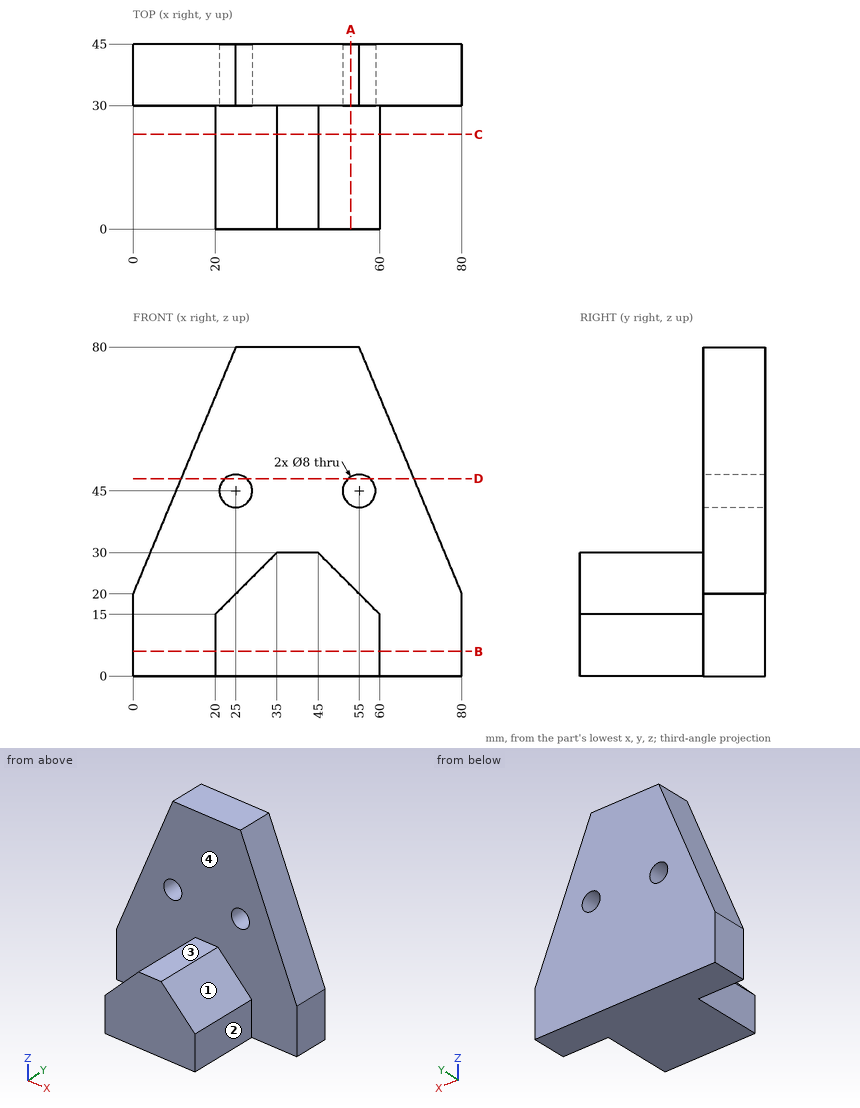
Study the drawing (mm; zero at the part's minimum x, y, z) and answer. A direction names the side the tool comes from. Round coordinates to 2 decimals unless told otherwise and drop trailing zeros. Order: outer loops, then holes, each group sorted by start corner. A loop starts at its lowest first (then second) coordinate and runs counter-clockwise, first axis right, second up. Notation, with made-up numbers: M 14.5,-39.5 L 47.5,-39.5 A24 cw 47.5,-11.5 Z; hole C 79.5,78.5 d9. An arc over 180 degrees is marked long. One line per item, written item: value.
Q1. For the marked faces 1, 2, 3 and 4, determine the directions among +Z, -Z, +X, -X, +Y, -Y from which every point of the face is accessible in a straight line to the end or side of a thin tool.
Derived:
face 1: +Z, +X, -Y
face 2: +Z, -Z, +X, -Y
face 3: +Z, +X, -X, -Y
face 4: +Z, -Y
Q2. Find section C-C on y = 23. Write down the section's boundary in (x, z).
Derived:
outline: M 20,0 L 60,0 L 60,15 L 45,30 L 35,30 L 20,15 Z
Q3. Find section D-D on z = 48. Write down the section's boundary in (x, y), then the cut area to 3 significant figures.
Derived:
outline: M 11.67,30 L 22.35,30 L 22.35,45 L 11.67,45 Z; M 27.65,30 L 52.35,30 L 52.35,45 L 27.65,45 Z; M 57.65,30 L 68.33,30 L 68.33,45 L 57.65,45 Z
area: 691 mm²
Q4. Flat-ended cylindrical pins translate along their axes: pin 1 (24 mm diameter, centred on x = 26, z = 57, fed in from -Y); pin 2 (4.5 mm diameter, centred on y = 8, z = 9.5, fed in from +X); pin 3 (4.5 mm diameter, centred on y = 8.5, z = 5.5, fed in from -X). Find the tip coordinate at first contact, or state that the pin passes through.
Derived:
pin 1: y = 30
pin 2: x = 60
pin 3: x = 20
Q5. Find section A-A on x = 53. Write down the section's boundary in (y, z).
Derived:
outline: M 0,0 L 45,0 L 45,41.54 L 30,41.54 L 30,22 L 0,22 Z; M 30,48.46 L 45,48.46 L 45,80 L 30,80 Z
Q6. Straight lines are drawn through the part: line 1 (X direction, y = 35, z = 45); line 2 (Y direction, x = 76, z = 5.5); line 3 (X direction, y = 9, z = 9). For each, find the intervals that lie inside material, in ascending order.
Derived:
line 1: 10.42 to 21, 29 to 51, 59 to 69.58
line 2: 30 to 45
line 3: 20 to 60
Q7. Find section B-B on z = 6. Write down the section's boundary in (x, y), then the cut area to 3 significant figures.
Derived:
outline: M 0,30 L 20,30 L 20,0 L 60,0 L 60,30 L 80,30 L 80,45 L 0,45 Z
area: 2,400 mm²
